```python
from build123d import *

# Parameters (mm, degrees)
SKETCH1_W                                            = 2300
SKETCH1_H                                            = 500
BOSS_EXTRUDE1_DEPTH                                  = 35
SKETCH2_R                                            = 40
CUT_EXTRUDE1_DEPTH                                   = 5
BOSS_EXTRUDE2_DEPTH                                  = 5
SKETCH4_R                                            = 2.5
CUT_EXTRUDE2_DEPTH                                   = 5
CUT_EXTRUDE3_DEPTH                                   = 1178.380567191
CHAMFER1_SIZE                                        = 10
SKETCH7_R                                            = 40
CUT_EXTRUDE4_DEPTH                                   = 5
CBORE_FOR_M6_HEXAGON_SOCKET_HEAD_CAP_SCR_D           = 6.6
CBORE_FOR_M6_HEXAGON_SOCKET_HEAD_CAP_SCR_CBORE_D     = 11
CBORE_FOR_M6_HEXAGON_SOCKET_HEAD_CAP_SCR_CBORE_DEPTH = 6.8
M8_TAPPED_HOLE1_D                                    = 6.8
M8_TAPPED_HOLE1_DEPTH                                = 19
M8_TAPPED_HOLE1_TIP                                  = 2.042926105


with BuildPart() as part:
    # Sketch1 → Boss-Extrude1 (new body)
    with BuildSketch(Plane.XY):
        Rectangle(SKETCH1_W, SKETCH1_H)
    extrude(amount=BOSS_EXTRUDE1_DEPTH)

    # Sketch2 → Cut-Extrude1 (cut)
    with BuildSketch(Plane(origin=(0, 0, 0), x_dir=(-1, 0, 0), z_dir=(0, 0, -1))):
        with Locations((-979, 2)):
            Circle(SKETCH2_R)
        with Locations((979, 2)):
            Circle(SKETCH2_R)
    extrude(amount=-CUT_EXTRUDE1_DEPTH, mode=Mode.SUBTRACT)

    # Sketch3 → Boss-Extrude2 (add)
    with BuildSketch(Plane(origin=(0, 0, 0), x_dir=(-1, 0, 0), z_dir=(0, 0, -1))):
        with BuildLine():
            Line((-947, -22), (-947, 26))
            ThreePointArc((-947, 26), (-939, 2), (-947, -22))
        make_face()
        with BuildLine():
            Line((947, -22), (947, 26))
            ThreePointArc((947, 26), (939, 2), (947, -22))
        make_face()
    extrude(amount=-BOSS_EXTRUDE2_DEPTH)

    # Sketch4 → Cut-Extrude2 (cut)
    with BuildSketch(Plane(origin=(0, 0, 5), x_dir=(-1, 0, 0), z_dir=(0, 0, -1))):
        with Locations((-947, -22)):
            Circle(SKETCH4_R)
        with Locations((-947, 26)):
            Circle(SKETCH4_R)
        with Locations((947, -22)):
            Circle(SKETCH4_R)
        with Locations((947, 26)):
            Circle(SKETCH4_R)
    extrude(amount=CUT_EXTRUDE2_DEPTH, mode=Mode.SUBTRACT)

    # Sketch6 → Cut-Extrude3 (cut, through all)
    with BuildSketch(Plane(origin=(0, 0, 0), x_dir=(-1, 0, 0), z_dir=(0, 0, -1))):
        with BuildLine():
            Line((1090, 30), (1190, 30))
            ThreePointArc((1190, 30), (1220, 0), (1190, -30))
            Line((1190, -30), (1090, -30))
            ThreePointArc((1090, -30), (1060, 0), (1090, 30))
        make_face()
        with BuildLine():
            Line((-1090, 30), (-1190, 30))
            ThreePointArc((-1190, 30), (-1220, 0), (-1190, -30))
            Line((-1190, -30), (-1090, -30))
            ThreePointArc((-1090, -30), (-1060, 0), (-1090, 30))
        make_face()
    extrude(amount=-CUT_EXTRUDE3_DEPTH, mode=Mode.SUBTRACT)

    # Chamfer1
    chamfer1_edges = [part.edges().sort_by_distance(p)[0] for p in [
        (-1150, 30, 17.5),
        (-1150, -30, 17.5),
        (1150, -30, 17.5),
        (1150, 30, 17.5),
        (1150, -250, 17.5),
        (-1150, -250, 17.5),
        (-1150, 250, 17.5),
        (1150, 250, 17.5),
    ]]
    chamfer(chamfer1_edges, length=CHAMFER1_SIZE)

    # Sketch7 → Cut-Extrude4 (cut)
    with BuildSketch(Plane(origin=(0, 0, 0), x_dir=(-1, 0, 0), z_dir=(0, 0, -1))):
        with Locations((340, -76)):
            Circle(SKETCH7_R)
        with Locations((397, 50)):
            Circle(SKETCH7_R)
        with Locations((-2.9799995, 46)):
            Circle(SKETCH7_R)
        with Locations((40, -76)):
            Circle(SKETCH7_R)
        with Locations((-259.958330439, -71)):
            Circle(SKETCH7_R)
        with Locations((-397, 46)):
            Circle(SKETCH7_R)
    extrude(amount=-CUT_EXTRUDE4_DEPTH, mode=Mode.SUBTRACT)

    # CBORE for M6 Hexagon socket head cap screws1 (through all)
    with Locations(Plane.XY.offset(35)):
        with Locations((-747, -8), (747, -8), (-979, 2), (979, 2)):
            CounterBoreHole(CBORE_FOR_M6_HEXAGON_SOCKET_HEAD_CAP_SCR_D / 2, CBORE_FOR_M6_HEXAGON_SOCKET_HEAD_CAP_SCR_CBORE_D / 2, CBORE_FOR_M6_HEXAGON_SOCKET_HEAD_CAP_SCR_CBORE_DEPTH)

    # M8 Tapped Hole1
    with Locations(Plane(origin=(0, 0, 0), x_dir=(-1, 0, 0), z_dir=(0, 0, -1))):
        with Locations((735.5, -125), (595.5, -125), (735.5, 124), (595.5, 124), (-604.5, -125), (-744.5, -125), (-604.5, 124), (-744.5, 124)):
            Hole(M8_TAPPED_HOLE1_D / 2, depth=M8_TAPPED_HOLE1_DEPTH)
            with Locations((0, 0, -(M8_TAPPED_HOLE1_DEPTH + M8_TAPPED_HOLE1_TIP / 2))):  # 118° drill point
                Cone(0, M8_TAPPED_HOLE1_D / 2, M8_TAPPED_HOLE1_TIP, mode=Mode.SUBTRACT)


solid = part.part
```
The model under review builds one solid part; all positions refer to its coordinate system, in mm. A direction names the side the tool comes from. Round coordinates to 2 decimals unless told otherwise and drop trailing zeros. Write each loop counter-clockwise with the first axis right and the second up, starting at its lowest first coordinate (ties: lowest second). Pieces come first, ordered by that corner, then holes. Notation, with made-up numbers: M -23.75,32 L 9.25,32 A27 ccw 9.25,50 Z; hole C 13.5,50.5 d7. An arc over 180 degrees is marked long. Use CSV: the item, a comma, the result in double quotes. Start each with the question number.
(1) We need section A-A, the plane x = -338. State the section outline as (y, z) points, then the cut area to 3 significant figures.
(2) The part is to be moulded in two halves that separate along X. For faces 1 (the face through (-16, 4, 0)), 2 (the face through (-396, 51, 5)), 3 (the face through (-39, -75, 5)), say which applies: +X half, -X half, draft (parallel to the pull), parting line (faces both ways), or undercut.
(3) For line 1 along X through (y, z) = (-125, 14); line 2 along Y through (x, z) = (604.5, 8.75); line 3 along Y through (x, z) = (-747, 30.75), list the stretches that pass through material, from the lowest coordinate up.
(4) We need section B-B, the plane x = 402. State the section outline as (y, z) points.
(5) Tool access review of faces 4 (the face through (-973, 3, 5)), 5 (the face through (-16, 4, 35)): name each direction out of +Z, -Z, +X, -X, +Y, -Y from which nothing blocks a thin tool from reaching the whole face with its end or side.
(6) Clearance check with flat-ended pins moving along their axes: P1, Ø5.5, axis at y = 7.5, z = 2.5, coming from the -X side; P2, Ø6, axis at x = -735.5, y = 124, coming from the -Z side; P3, Ø5.5, axis at y = 12, z = 3, coming from the +X side. State where each tip first meets the part, or that it passes through.
Findings:
1,outline,"M -250,0 L -115.95,0 L -115.95,5 L -36.05,5 L -36.05,0 L 250,0 L 250,35 L -250,35 Z"
1,area,"17,100 mm^2"
2,face 1,"draft"
2,face 2,"undercut"
2,face 3,"undercut"
3,line 1,"-1150 to -738.9, -732.1 to -598.9, -592.1 to 601.1, 607.9 to 741.1, 747.9 to 1150"
3,line 2,"-250 to -128.4, -121.6 to 120.6, 127.4 to 250"
3,line 3,"-250 to -13.5, -2.5 to 250"
4,outline,"M -250,0 L 6.31,0 L 6.31,5 L 85.69,5 L 85.69,0 L 250,0 L 250,35 L -250,35 Z"
5,face 4,"-Z"
5,face 5,"+Z, +X, -X, +Y, -Y"
6,P1,"x = -1061.81"
6,P2,"z = 19.24"
6,P3,"x = 1063.88"
